Study the drawing (mm; zero at the part's minimum x, y, z) and answer. Coordinates: 2 decimals unless noted, no trailing zeros. Loops run counter-clockwise (first coordinate to the right, second up) from the corner with the lowest first, then second, coordinate; pieces in that order, holes last. Notation, with made-up numbers: M 64.5,18.25 L 99.5,18.25 A23 cw 99.5,55.25 Z; hole C -39.75,76 d5. An arc over 180 degrees is marked long. Use one line per item in the form item = value. Start each with the question number.
1. The part is cut by section B-B (y = 5.5). Give the number of separate pieces and of enclosed holes in the cut face, plus the area to 3 significant figures.
2. The part is cut by section A-A (z = 108). Give the vertices of the cut face in (x, y), plus the area to 3 significant figures.
3. Find the intervals of material crossed by probe 1 along X at (y, z) = (1.25, 190); probe 2 along X at (y, z) = (7.5, 425); probe 3 along Z at (x, y) = (169.5, 5.25), in increasing order. Write a range as [from, to].
4. Flat-ended cylindrical pins translate along their axes: pin 1 (5 mm diameter, centred on x = 60, z = 75, fed in from +Y); pin 2 (1 mm diameter, centred on y = 4.5, z = 441.5, fed in from -X); pin 3 (1 mm diameter, centred on x = 39.5, y = 10, fed in from -Z). Find the tip coordinate at first contact, or state that the pin passes through.
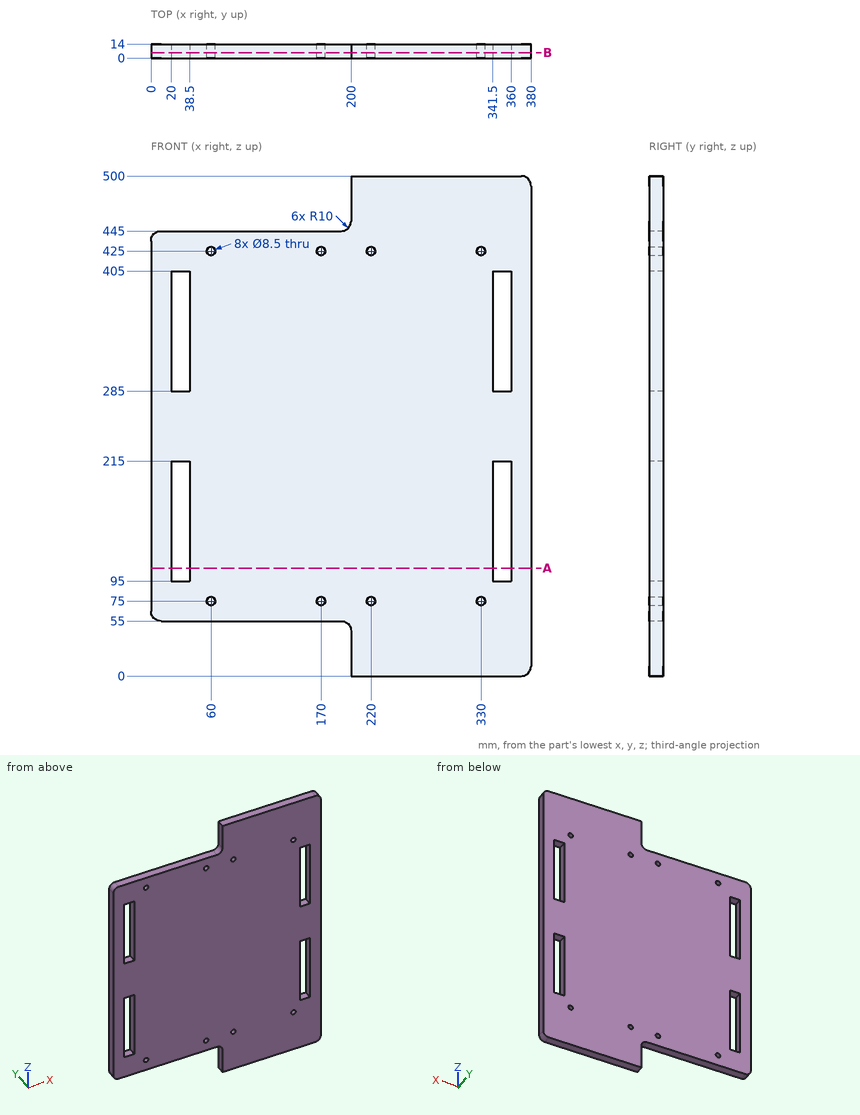
Computed values:
q1.separate_pieces = 1
q1.enclosed_holes = 12
q1.area = 159,000 mm²
q2.outline = M 0,0 L 20,0 L 20,14 L 0,14 Z; M 38.5,0 L 341.5,0 L 341.5,14 L 38.5,14 Z; M 360,0 L 380,0 L 380,14 L 360,14 Z
q2.area = 4,800 mm²
q3.probe_1 = [0, 20], [38.5, 341.5], [360, 380]
q3.probe_2 = [0, 55.75], [64.25, 165.75], [174.25, 215.75], [224.25, 325.75], [334.25, 380]
q3.probe_3 = [55, 70.78], [79.22, 420.78], [429.22, 445]
q4.pin_1 = through
q4.pin_2 = 2
q4.pin_3 = 55
